Geometry check sheet. Reference: the model listing, model coordinates, mm. A direction names the side the tool comes from. Coordinates: 2 decimals unless noted, no trailing zeros. Write each loop counter-clockwise with the first axis right and the second up, starting at its lowest first coordinate (ties: lowest second). Pieces come first, ordered by that corner, then holes. Notation, with made-up numbers: M -31.75,40.25 L -26.75,40.25 A27 cw -26.75,65.25 Z; hole C -19,35.5 d10. An arc over 180 degrees is marked long. Answer as a JSON object with one key per item and string values. Group by question number.
```python
from build123d import *
from build123d.topology import SkipClean

# Parameters (mm, degrees)
SKETCH_1_2_R                   = 4
BOSS_EXTRUDE1_DEPTH            = 9.7
BOSS_EXTRUDE2_DEPTH            = 4
BOSS_EXTRUDE3_START            = 13.7
SKETCH_1_2_2_R                 = 4
BOSS_EXTRUDE3_DEPTH            = 20
SKETCH3_R                      = 2
BOSS_EXTRUDE4_DEPTH            = 12
CHAMFER1_SIZE                  = 0.5
CUT_EXTRUDE1_DEPTH             = 12
F_3_2_3_2_DIAMETER_HOLE1_D     = 3.2
F_3_2_3_2_DIAMETER_HOLE1_DEPTH = 14
F_3_2_3_2_DIAMETER_HOLE1_TIP   = 0.96137699
F_3_2_3_2_DIAMETER_HOLE2_D     = 3.2
F_3_2_3_2_DIAMETER_HOLE2_DEPTH = 2.499
F_3_2_3_2_DIAMETER_HOLE2_TIP   = 0.96137699


with BuildPart() as part:
    # Sketch 1_2 → Boss-Extrude1 (new body)
    with BuildSketch(Plane.XY):
        Circle(SKETCH_1_2_R)
    extrude(amount=BOSS_EXTRUDE1_DEPTH)

    # Sketch2 → Boss-Extrude2 (add)
    with SkipClean():  # the faces are left unmerged after this step: merging them gives an invalid solid
        with BuildSketch(Plane.XY.offset(9.7)):
            with BuildLine():
                Line((-3.872983346, 1), (-2.1, 2.5))
                Line((-2.1, 2.5), (2.1, 2.5))
                Line((2.1, 2.5), (3.708099244, 1.5))
                ThreePointArc((3.708099244, 1.5), (3.957811022, -0.579423775), (3.122498999, -2.5))
                Line((3.122498999, -2.5), (-3.122498999, -2.5))
                ThreePointArc((-3.122498999, -2.5), (-3.911098735, -0.838633823), (-3.872983346, 1))
            make_face()
        extrude(amount=BOSS_EXTRUDE2_DEPTH)

    # Sketch 1_2 2 → Boss-Extrude3 (add)
    with SkipClean():  # the faces are left unmerged after this step: merging them gives an invalid solid
        with BuildSketch(Plane.XY.offset(BOSS_EXTRUDE3_START)):
            Circle(SKETCH_1_2_2_R)
        extrude(amount=BOSS_EXTRUDE3_DEPTH)

    # Sketch3 → Boss-Extrude4 (add)
    with SkipClean():  # the faces are left unmerged after this step: merging them gives an invalid solid
        with BuildSketch(Plane.XY.offset(33.7)):
            Circle(SKETCH3_R)
        extrude(amount=BOSS_EXTRUDE4_DEPTH)

    # Chamfer1
    chamfer1_edges = [part.edges().sort_by_distance(p)[0] for p in [
        (-2, 0, 45.7),
    ]]
    chamfer(chamfer1_edges, length=CHAMFER1_SIZE)

    # Sketch4 → Cut-Extrude1 (cut)
    with SkipClean():  # the faces are left unmerged after this step: merging them gives an invalid solid
        with BuildSketch(Plane.XY.offset(9.7)):
            with BuildLine():
                Line((3.122498999, -2.5), (-3.122498999, -2.5))
                ThreePointArc((-3.122498999, -2.5), (0, -4), (3.122498999, -2.5))
            make_face()
        extrude(amount=CUT_EXTRUDE1_DEPTH, mode=Mode.SUBTRACT)

    # Ø3.2 (3.2) Diameter Hole1
    with Locations(Plane(origin=(0, 0, 0), x_dir=(-1, 0, 0), z_dir=(0, 0, -1))):
        with Locations((0, 0)):
            Hole(F_3_2_3_2_DIAMETER_HOLE1_D / 2, depth=F_3_2_3_2_DIAMETER_HOLE1_DEPTH)
            with Locations((0, 0, -(F_3_2_3_2_DIAMETER_HOLE1_DEPTH + F_3_2_3_2_DIAMETER_HOLE1_TIP / 2))):  # 118° drill point
                Cone(0, F_3_2_3_2_DIAMETER_HOLE1_D / 2, F_3_2_3_2_DIAMETER_HOLE1_TIP, mode=Mode.SUBTRACT)

    # Ø3.2 (3.2) Diameter Hole2
    with Locations(Plane(origin=(-0.020216214, 2.5, 11.7), x_dir=(0, 0, 1), z_dir=(0, 1, 0))):
        with Locations((0, 0)):
            Hole(F_3_2_3_2_DIAMETER_HOLE2_D / 2, depth=F_3_2_3_2_DIAMETER_HOLE2_DEPTH)
            with Locations((0, 0, -(F_3_2_3_2_DIAMETER_HOLE2_DEPTH + F_3_2_3_2_DIAMETER_HOLE2_TIP / 2))):  # 118° drill point
                Cone(0, F_3_2_3_2_DIAMETER_HOLE2_D / 2, F_3_2_3_2_DIAMETER_HOLE2_TIP, mode=Mode.SUBTRACT)


solid = part.part
```
1) Draft check along Z on faces 1 (the conical face through (0.278, 0.012, 14.794)), 2 (the flat face through (0, 3, 13.7)), 3 (the flat face through (-2, -1, 33.7)), 4 (the cylindrical face through (0, -2, 39)). Enter one of: +Z half, -Z half, draft (parallel to the pull), parting line (faces both ways), or undercut.
2) Set-up check for faces 5 (the flat face through (-1, 2.5, 10)), 6 (the flat face through (-3, 1.74, 11.67)), 7 (the flat face through (0, -3, 21.7)): record each of +Z, -Z, +X, -X, +Y, -Y from which the full face is reachable in a straight line by a thin tool's end or side.
3) Go/stop test with flat-tipped pins: pin 1 Ø2 at (x, z) = (0.5, 11) entering from +Y; pin 2 Ø1.5 at (x, y) = (0, 2.5) entering from +Z; pin 3 Ø2 at (y, z) = (-3, 29) entering from -X. Record where each tip stops, or that it passes through.
4) Section check A-A (y = 3.25). Record the cut outline in (x, z), then the cut area to 3 significant figures.
5) Material ranges on probe 1 along X at (y, z) = (0, 4.5); probe 2 along Z at (x, y) = (-0.75, 3), recorded low to high. Write a range as [from, to].
6) Section check B-B (z = 39.5). Record the cut outline in (x, y), then the cut area to 3 significant figures.
Entries:
{
 "1": {"face 1": "-Z half", "face 2": "undercut", "face 3": "+Z half", "face 4": "draft"},
 "2": {"face 5": "+X, -X, +Y", "face 6": "-X, +Y", "face 7": "+X, -X, -Y"},
 "3": {"pin 1": "y = 2.5", "pin 2": "z = 45.45", "pin 3": "x = -3.46"},
 "4": {"outline": "M -2.33,0 L 2.33,0 L 2.33,9.7 L -2.33,9.7 Z; M -2.33,13.7 L 2.33,13.7 L 2.33,33.7 L -2.33,33.7 Z", "area": "139 mm^2"},
 "5": {"probe 1": "[-4, -1.6], [1.6, 4]", "probe 2": "[0, 9.7], [13.7, 33.7]"},
 "6": {"outline": "C 0,0 d4", "area": "12.6 mm^2"}
}
